Geometry check sheet. Reference: the model listing, model coordinates, mm. Coordinates: 2 decimals unless noted, no trailing zeros. Order: outer loops, then holes, each group sorted by start corner. A loop starts at its lowest first (then second) coordinate and runs counter-clockwise, first axis right, second up. Notation, with made-up numbers: M -3.5,83 L 7.5,83 A13 cw 7.5,95 Z; hole C 9.25,69 d2. An arc over 180 degrees is marked long. One line per item, written item: value. Start each with the question number.
1) Sectioned sample at A-A, the plane x = 0. Enter the section's corners in (y, z).
2) Sectioned sample at D-D, the plane x = 52.5. Enter the section's corners in (y, z).
3) Go/stop test with flat-tipped pins: P1, Ø23.5, axis at x = 0, y = 0, coming from the +Z side; P2, Ø1.5, axis at x = 16.5, z = -18, coming from the -Y side; P3, Ø5.5, axis at x = 16, z = -4, coming from the +Y side; P4, Ø1.2, axis at y = 1, z = -32.5, coming from the -X side. Record where each tip stops, or that it passes through.
4) Sectioned sample at B-B, the plane y = -10. Enter the section's corners in (x, z), then the cut area to 3 significant figures.
5) Sectioned sample at C-C, the plane z = -14. Enter the section's corners in (x, y), then the cut area to 3 significant figures.
6) Thickness scan on L1, parallel to Y at x = 0, z = -7; L2, parallel to Z at x = 46.5, y = -24.5; L3, parallel to Z at x = 57.5, y = 19.5. Record the ranges inside material, lowest first. Write a range as from..to.
```python
from build123d import *
from build123d.topology import SkipClean

# Parameters (mm, degrees)
ARM_PLATE_DEPTH        = 10
HUB_START              = -20
HUB_BOSS_PROFILE_R     = 22
HUB_BOSS_PROFILE_R_2   = 7.5
HUB_BOSS_DEPTH         = 20
ARM_HOLE_DEPTH         = 95.498677239
ARM_HOLE_DEPTH_BACK    = 95.498677239
ARM_HOLE_PROFILE_R     = 7.5
HUB_HOUSING_PROFILE_R  = 31
HUB_HOUSING_DEPTH      = 40
KEYED_BORE_DEPTH       = 101.647901121
KEYED_BORE_DEPTH_BACK  = 101.647901121
ANGLED_ARM_PROFILE_R   = 7.5
ANGLED_ARM_PLATE_DEPTH = 10


with BuildPart() as part:
    # Arm Plate Profile → Arm Plate (new body)
    with BuildSketch(Plane.XY):
        with BuildLine():
            Line((4.292307692, 30.701402161), (68.046153846, 21.788091856))
            ThreePointArc((68.046153846, 21.788091856), (87, 0), (68.046153846, -21.788091856))
            Line((68.046153846, -21.788091856), (4.292307692, -30.701402161))
            ThreePointArc((4.292307692, -30.701402161), (-31, 0), (4.292307692, 30.701402161))
        make_face()
    extrude(amount=-ARM_PLATE_DEPTH)

    # Hub Boss Profile → Hub Boss (add)
    with SkipClean():  # the faces are left unmerged after this step: merging them gives an invalid solid
        with BuildSketch(Plane(origin=(0, 0, -10), x_dir=(-1, 0, 0), z_dir=(0, 0, -1)).offset(HUB_START)):
            with Locations(Location((-65, 0, 0), (0, 0, 262.041168118))):
                Circle(HUB_BOSS_PROFILE_R)
            with Locations((-65, 0)):
                Circle(HUB_BOSS_PROFILE_R_2, mode=Mode.SUBTRACT)
        extrude(amount=HUB_BOSS_DEPTH)

    # Arm Hole Profile → Arm Hole (cut, two sides: drawn at the far end of the back side and taken through both)
    with SkipClean():  # the faces are left unmerged after this step: merging them gives an invalid solid
        with BuildSketch(Plane(origin=(0, 0, -10), x_dir=(-1, 0, 0), z_dir=(0, 0, -1)).offset(-ARM_HOLE_DEPTH_BACK)):
            with Locations((-65, 0)):
                Circle(ARM_HOLE_PROFILE_R)
        extrude(amount=ARM_HOLE_DEPTH + ARM_HOLE_DEPTH_BACK, mode=Mode.SUBTRACT)

    # Hub Housing Profile → Hub Housing (add)
    with SkipClean():  # the faces are left unmerged after this step: merging them gives an invalid solid
        with BuildSketch(Plane(origin=(0, 0, -10), x_dir=(-1, 0, 0), z_dir=(0, 0, -1))):
            with Locations(Location((0, 0, 0), (0, 0, 97.958831882))):
                Circle(HUB_HOUSING_PROFILE_R)
            with BuildLine():
                Line((-12.845232579, -2), (-18, -2))
                Line((-18, -2), (-18, 2))
                Line((-18, 2), (-12.845232579, 2))
                ThreePointArc((-12.845232579, 2), (13, 0), (-12.845232579, -2))
            make_face(mode=Mode.SUBTRACT)
        extrude(amount=HUB_HOUSING_DEPTH)

    # Keyed Bore Profile → Keyed Bore (cut, two sides: drawn at the far end of the back side and taken through both)
    with SkipClean():  # the faces are left unmerged after this step: merging them gives an invalid solid
        with BuildSketch(Plane(origin=(0, 0, -10), x_dir=(-1, 0, 0), z_dir=(0, 0, -1)).offset(-KEYED_BORE_DEPTH_BACK)):
            with BuildLine():
                Line((-18, -2), (-12.845232579, -2))
                ThreePointArc((-12.845232579, -2), (13, 0), (-12.845232579, 2))
                Line((-12.845232579, 2), (-18, 2))
                Line((-18, 2), (-18, -2))
            make_face()
        extrude(amount=KEYED_BORE_DEPTH + KEYED_BORE_DEPTH_BACK, mode=Mode.SUBTRACT)

    # Angled Arm Profile → Angled Arm Plate (add)
    with SkipClean():  # the faces are left unmerged after this step: merging them gives an invalid solid
        with BuildSketch(Plane.XY.offset(-50)):
            with BuildLine():
                Line((-17.469853837, 25.608674447), (-116.321009242, -41.826102006))
                ThreePointArc((-116.321009242, -41.826102006), (-122.975607337, -71), (-94.382971499, -79.823897994))
                Line((-94.382971499, -79.823897994), (13.442835709, -27.933674447))
                ThreePointArc((13.442835709, -27.933674447), (26.846787517, 15.5), (-17.469853837, 25.608674447))
            make_face()
            with Locations((-103.923048454, -60)):
                Circle(ANGLED_ARM_PROFILE_R, mode=Mode.SUBTRACT)
            with BuildLine():
                Line((18, -2), (18, 2))
                Line((18, 2), (12.845232579, 2))
                ThreePointArc((12.845232579, 2), (-13, 0), (12.845232579, -2))
                Line((12.845232579, -2), (18, -2))
            make_face(mode=Mode.SUBTRACT)
        extrude(amount=-ANGLED_ARM_PLATE_DEPTH)


solid = part.part
```
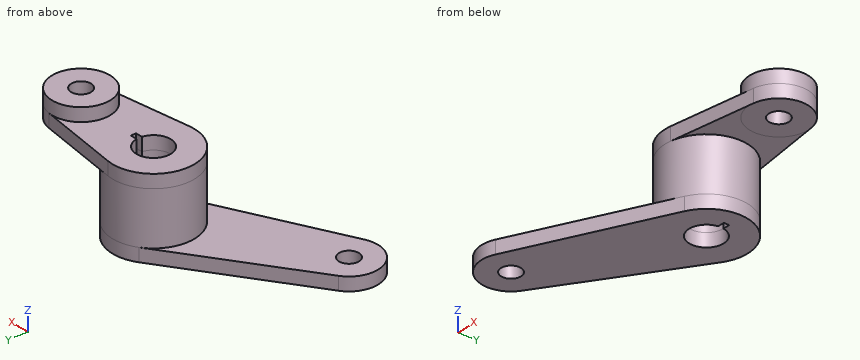
Final values:
1. outline: M -34.4,-60 L -13,-60 L -13,0 L -31,0 L -31,-50 L -34.4,-50 Z; M 13,-60 L 31,-60 L 31,0 L 13,0 Z
2. outline: M -23.96,-10 L 23.96,-10 L 23.96,0 L 18.1,0 L 18.1,10 L -18.1,10 L -18.1,0 L -23.96,0 Z
3. P1: passes through
3. P2: stops at y = -26.7
3. P3: stops at y = 29.45
3. P4: stops at x = -31
4. outline: M -69.67,-60 L -8.31,-60 L -8.31,0 L -29.34,0 L -29.34,-50 L -69.67,-50 Z; M 8.31,-60 L 29.34,-60 L 29.34,-10 L 84.6,-10 L 84.6,10 L 45.4,10 L 45.4,0 L 8.31,0 Z
4. area: 3,870 mm^2
5. outline: C 0,0 d62; hole M 12.85,-2 L 18,-2 L 18,2 L 12.85,2 A13 ccw long Z
5. area: 2,470 mm^2
6. L1: y = -31..-13, 13..31
6. L2: z = -10..0
6. L3: z = -10..10
